from build123d import *

# Parameters (mm, degrees)
BRACKET_PROFILE_SKETCH_W = 35
BRACKET_PROFILE_SKETCH_H = 80
BRACKET_BODY_DEPTH       = 30
SIDE_RELIEF_CUT_DEPTH    = 62.032778079
RING_BOSS_DEPTH          = 8
BOSS_BORE_SKETCH_R       = 8
BOSS_BORE_16_DEPTH       = 8
BASE_HOLES_SKETCH_R      = 5
BASE_HOLES_DEPTH         = 79.14249804
EDGE_FILLET_R5_R         = 5
TOP_SLOT_CUT_DEPTH       = 47.853495067


with BuildPart() as part:
    # Bracket Profile Sketch → Bracket Body (new body)
    with BuildSketch(Plane(origin=(0, 0, 0), x_dir=(0, 0, -1), z_dir=(1, 0, 0))):
        Rectangle(BRACKET_PROFILE_SKETCH_W, BRACKET_PROFILE_SKETCH_H)
    extrude(amount=BRACKET_BODY_DEPTH)

    # Side Relief Sketch → Side Relief Cut (cut, through all)
    with BuildSketch(Plane.XY.offset(17.5)):
        Polygon((13, 40), (13, 20), (8.358661264, 20), (8.358661264, -30), (30, -30), (30, 40), align=None)
    extrude(amount=-SIDE_RELIEF_CUT_DEPTH, mode=Mode.SUBTRACT)

    # Ring Boss Sketch → Ring Boss (add)
    with BuildSketch(Plane(origin=(8.358661264, 0, 0), x_dir=(0, 0, -1), z_dir=(1, 0, 0))):
        with BuildLine():
            Line((-3, -30), (3, -30))
            Line((3, -30), (3, -23.162446581))
            ThreePointArc((3, -23.162446581), (0, 3.5), (-3, -23.162446581))
            Line((-3, -23.162446581), (-3, -30))
        make_face()
    extrude(amount=RING_BOSS_DEPTH)

    # Boss Bore Sketch → Boss Bore Ø16 (cut)
    with BuildSketch(Plane(origin=(16.358661264, 0, 0), x_dir=(0, 0, -1), z_dir=(1, 0, 0))):
        with Locations(Location((0, -10, 0), (0, 0, 90))):
            Circle(BOSS_BORE_SKETCH_R)
    extrude(amount=-BOSS_BORE_16_DEPTH, mode=Mode.SUBTRACT)

    # Base Holes Sketch → Base Holes (cut, through all)
    with BuildSketch(Plane(origin=(0, -30, 0), x_dir=(1, 0, 0), z_dir=(0, 1, 0))):
        with Locations(Location((22, 10.5, 0), (0, 0, 180))):
            Circle(BASE_HOLES_SKETCH_R)
        with Locations((22, -10.5)):
            Circle(BASE_HOLES_SKETCH_R)
    extrude(amount=-BASE_HOLES_DEPTH, mode=Mode.SUBTRACT)

    # Edge Fillet R5
    edge_fillet_r5_edges = [part.edges().sort_by_distance(p)[0] for p in [
        (6.5, 40, 17.5),
        (6.5, 40, -17.5),
    ]]
    fillet(edge_fillet_r5_edges, radius=EDGE_FILLET_R5_R)

    # Top Slot Sketch → Top Slot Cut (cut, through all)
    with BuildSketch(Plane(origin=(13, 0, 0), x_dir=(0, 0, -1), z_dir=(1, 0, 0))):
        with BuildLine():
            Line((-5.180950854, 35), (5.819049146, 35))
            ThreePointArc((5.819049146, 35), (10.819049146, 30), (5.819049146, 25))
            Line((5.819049146, 25), (-5.180950854, 25))
            ThreePointArc((-5.180950854, 25), (-10.180950854, 30), (-5.180950854, 35))
        make_face()
    extrude(amount=-TOP_SLOT_CUT_DEPTH, mode=Mode.SUBTRACT)


solid = part.part
Input: part model. Units: mm. Frame: model coordinates. A direction names the side the tool comes from. Round coordinates to 2 decimals unless told otherwise and drop trailing zeros. Loops run counter-clockwise (first coordinate to the right, second up) from the corner with the lowest first, then second, coordinate; pieces in that order, holes last. Notation, with made-up numbers: M 8.25,12.5 L 12.25,12.5 A32 cw 12.25,42.5 Z; hole C -32.75,62.25 d1. An arc over 180 degrees is marked long. Answer as CSV lines item,"result". Start each with the question number.
(1) Section D-D, the plane z = 0. Output: boundary loops of the cut face in (x, y), plus the area to 3 significant figures.
(2) Section C-C, the plane x = 22. Output: boundary loops of the cut face in (y, z), plus the area to 3 significant figures.
(3) Draft query along Y for faces 6 (the cylindrical face through (6.59, 29.89, 10.18)), 7 (the cylindrical face through (6.59, 38.57, -16)), 8 (the cylindrical face through (26.995, -34.93, -10.28)). Return one class per face: released by +Y, released by -Y, zero draft, split by the parting line, or undercut.
(4) Line query: line 1 (Z direction, x = 22, y = -36.25); line 2 (Z direction, x = 19, y = -37); line 3 (Z direction, x = 10.25, y = -10). Output: solid intervals per line, ascending. Write a range as [from, to].
(5) Section A-A, the plane x = 9.25. Output: boundary loops of the cut face in (y, z), plus the area to 3 significant figures.
(6) First-contact query: pin 1 (12 mm diameter, centred on y = -22, z = 5.5, fed in from -X); pin 2 (6 mm diameter, centred on y = 26, z = -12, fed in from +X); pin 3 (8 mm diameter, centred on x = 22, z = -10.5, fed in from +Y); pin 4 (3.5 mm diameter, centred on x = 13, y = -27, fed in from -Z). Flat tips, straight axial feed; report the tip coordinate or a pass-through.
(7) Reachability of faces 1 (the flat face through (16.359, -17, -6)), 2 (the cylindrical face through (12.41, -11.73, -7.81)), 3 (the flat face through (6, 40, 0)), 4 (the cylindrical face through (6.591, 30.11, -10.818)), 5 (the flat face through (12, -27, 3)) from +Z, -Z, +X, -X, +Y, -Y: full face, straight path, thin tool, end or side. Return the list, or none.
(8) Section B-B, the plane y = 30. Output: boundary loops of the cut face in (x, z).
Values found:
1,outline,"M 0,-40 L 30,-40 L 30,-30 L 16.36,-30 L 16.36,-18 L 8.36,-18 L 8.36,-2 L 16.36,-2 L 16.36,3.5 L 8.36,3.5 L 8.36,20 L 13,20 L 13,25 L 0,25 Z; M 0,35 L 13,35 L 13,40 L 0,40 Z"
1,area,"988 mm²"
2,outline,"M -40,-17.5 L -30,-17.5 L -30,-15.5 L -40,-15.5 Z; M -40,-5.5 L -30,-5.5 L -30,5.5 L -40,5.5 Z; M -40,15.5 L -30,15.5 L -30,17.5 L -40,17.5 Z"
2,area,"150 mm²"
3,face 6,"undercut"
3,face 7,"released by +Y"
3,face 8,"zero draft"
4,line 1,"z = [-17.5, -15.5], [-5.5, 5.5], [15.5, 17.5]"
4,line 2,"z = [-17.5, -14.5], [-6.5, 6.5], [14.5, 17.5]"
4,line 3,"z = [-13.5, -8], [8, 13.5]"
5,outline,"M -40,-17.5 L -30,-17.5 L -30,-3 L -23.16,-3 A13.5 ccw long -23.16,3 L -30,3 L -30,17.5 L -40,17.5 Z; M 20,-17.5 L 35,-17.5 A5 ccw 40,-12.5 L 40,12.5 A5 ccw 35,17.5 L 20,17.5 Z; hole C -10,0 d16; hole M 25,-5.82 A5 ccw 35,-5.82 L 35,5.18 A5 ccw 25,5.18 Z"
5,area,"1,260 mm²"
6,pin 1,"stops at x = 0"
6,pin 2,"stops at x = 13"
6,pin 3,"passes through"
6,pin 4,"stops at z = -3"
7,face 1,"+Z, -Z, +X, +Y"
7,face 2,"+X"
7,face 3,"+Z, -Z, +X, -X, +Y"
7,face 4,"+X, -X"
7,face 5,"+Z, +X"
8,outline,"M 0,-17.5 L 13,-17.5 L 13,-10.82 L 0,-10.82 Z; M 0,10.18 L 13,10.18 L 13,17.5 L 0,17.5 Z"
